from build123d import *

# Parameters (mm, degrees)
BASE_PLATE_PROFILE_SKETCH_R   = 6
BASE_PLATE_PROFILE_SKETCH_R_2 = 5
BASE_PLATE_PROFILE_SKETCH_R_3 = 9.5
BASE_PLATE_14MM_DEPTH         = 14
INTERLOCKING_RAILS_SKETCH_W   = 89
INTERLOCKING_RAILS_SKETCH_H   = 9
INTERLOCKING_RAILS_SKETCH_W_2 = 27
INTERLOCKING_RAILS_SKETCH_H_2 = 19
INTERLOCKING_RAILS_SKETCH_W_3 = 18
INTERLOCKING_RAILS_32MM_DEPTH = 32
RAIL_SLOT_CUT_REACH           = 205.941


with BuildPart() as part:
    # Base Plate Profile Sketch → Base Plate 14mm (new body)
    with BuildSketch(Plane(origin=(0, 0, 0), x_dir=(1, 0, 0), z_dir=(0, 1, 0))):
        with BuildLine():
            Line((0, 0), (-117.109003688, 0))
            ThreePointArc((-117.109003688, 0), (-123.536879785, 2.339555569), (-126.957081218, 8.263518223))
            Line((-126.957081218, 8.263518223), (-139.9366539, 81.874332802))
            ThreePointArc((-139.9366539, 81.874332802), (-135.998914322, 96.570176974), (-122.210114346, 103))
            Line((-122.210114346, 103), (-56.522720755, 103))
            ThreePointArc((-56.522720755, 103), (-49.311103576, 105.408723877), (-44.994618812, 111.667903721))
            Line((-44.994618812, 111.667903721), (-38.331477751, 134.720469728))
            ThreePointArc((-38.331477751, 134.720469728), (-19.616213283, 146.832039713), (-5, 130))
            Line((-5, 130), (-5, 77.5))
            Line((-5, 77.5), (0, 55))
            Line((0, 55), (0, 0))
        make_face()
        with Locations(Location((-22, 130, 0), (0, 0, 270))):
            Circle(BASE_PLATE_PROFILE_SKETCH_R, mode=Mode.SUBTRACT)
        with Locations(Location((-122.210114346, 85, 0), (0, 0, 270))):
            Circle(BASE_PLATE_PROFILE_SKETCH_R_2, mode=Mode.SUBTRACT)
        with Locations(Location((-90.210114346, 79.5, 0), (0, 0, 270))):
            Circle(BASE_PLATE_PROFILE_SKETCH_R_3, mode=Mode.SUBTRACT)
        with Locations(Location((-28.210114346, 79.5, 0), (0, 0, 270))):
            Circle(BASE_PLATE_PROFILE_SKETCH_R_3, mode=Mode.SUBTRACT)
    extrude(amount=BASE_PLATE_14MM_DEPTH)

    # Interlocking Rails Sketch → Interlocking Rails 32mm (add)
    with BuildSketch(Plane(origin=(0, 0, 0), x_dir=(1, 0, 0), z_dir=(0, 1, 0))):
        with Locations((-49.5, 4.5)):
            Rectangle(INTERLOCKING_RAILS_SKETCH_W, INTERLOCKING_RAILS_SKETCH_H)
        with Locations((-80.5, 27.5)):
            Rectangle(INTERLOCKING_RAILS_SKETCH_W_2, INTERLOCKING_RAILS_SKETCH_H_2)
        with Locations((-49.5, 50.5)):
            Rectangle(INTERLOCKING_RAILS_SKETCH_W, INTERLOCKING_RAILS_SKETCH_H)
        with Locations((-4.5, 27.5)):
            Rectangle(INTERLOCKING_RAILS_SKETCH_W_3, INTERLOCKING_RAILS_SKETCH_H_2)
    extrude(amount=INTERLOCKING_RAILS_32MM_DEPTH)

    # Rail Slot Sketch → Rail Slot Cut (cut, up to next)
    with BuildSketch(Plane(origin=(0, 14, 0), x_dir=(1, 0, 0), z_dir=(0, 1, 0)), mode=Mode.PRIVATE) as rail_slot_cut_sk1:
        Polygon((-81.5, 46), (-81.5, 37), (-67, 37), (-67, 18), (-81.5, 18), (-81.5, 9), (-21.5, 9), (-21.5, 46), align=None)
    rail_slot_cut_tool1 = extrude(rail_slot_cut_sk1.sketch, amount=-RAIL_SLOT_CUT_REACH, mode=Mode.PRIVATE) & part.part
    add(rail_slot_cut_tool1.solids().sort_by_distance((-48.276742, 14, -27.5))[0], mode=Mode.SUBTRACT)


solid = part.part
Could you check a few things on this model? Use its own coordinates, in mm. A direction names the side the tool comes from. Coordinates: 2 decimals unless noted, no trailing zeros. Order: outer loops, then holes, each group sorted by start corner. A loop starts at its lowest first (then second) coordinate and runs counter-clockwise, first axis right, second up.
Q1. Suppose I cut it at A-A on y = 24. Please give me the cut outline in (x, z).
Q2. Please list where these lines run through material, in increasing order: L1, parallel to Z at x = -72.5, y = 7.5; L2, parallel to Z at x = -71, y = 16.5; L3, parallel to Z at x = -50, y = 21.
Q3. Which directions (+Z, -Z, +X, -X, +Y, -Y) give clear straight access to the entire face, cutting with the end or side of a thin tool? Please do faces 1 (the flat face through (-94, 23, -4)), 2 (the flat face through (-5, 23, -4)), 3 (the flat face through (-50, 16, -46)).
Q4. Suppose I cut it at B-B on z = -42.5. Please give me the cut outline in (x, y), and give its area (3 significant figures).
Q5. Suppose I cut it at C-C on x = -52. Please give me the cut outline in (y, z).
Q6. Thinking about a two-plate mould opening in X: for faces 4 (the cylindrical face through (-19.954, 6.902, -146.876)), 5 (the flat face through (-50, 16, -9)), 6 (the flat face through (4.5, 16, -27)), which applies, released by +X, released by -X, zero draft, split by the parting line, or undercut?
Q7. Suppose I cut it at D-D on z = -85. Please give me the cut outline in (x, y), and give its area (3 significant figures).
Q8. Will these pins go through, and if not, where does the flat tip stop? pin 1 (1.5 mm diameter, centred on x = -14, z = -106, fed in from +Y); pin 2 (4.5 mm diameter, centred on y = 23, z = -48.5, fed in from +X); pin 3 (10 mm diameter, centred on x = -24.5, y = 13, fed in from +Z); pin 4 (15.5 mm diameter, centred on y = 6, z = -6, fed in from +X).
Answer:
1. outline: (-94, -55) - (-5, -55) - (-5, -46) - (-94, -46) - close; (-94, -37) - (-67, -37) - (-67, -18) - (-94, -18) - close; (-94, -9) - (-5, -9) - (-5, 0) - (-94, 0) - close; (-13.5, -37) - (4.5, -37) - (4.5, -18) - (-13.5, -18) - close
2. L1: z = -103 to -46, -37 to -18, -9 to 0
2. L2: z = -55 to -46, -37 to -18, -9 to 0
2. L3: z = -55 to -46, -9 to 0
3. face 1: +Z, -Z, -X, +Y
3. face 2: +Z, +X, +Y
3. face 3: +Y
4. outline: (-132.99, 0) - (-81.5, 0) - (-81.5, 14) - (-132.99, 14) - close; (-21.5, 0) - (0, 0) - (0, 14) - (-21.5, 14) - close
4. area: 1,020 mm2
5. outline: (0, -103.88) - (14, -103.88) - (14, -55) - (32, -55) - (32, -46) - (0, -46) - close; (0, -9) - (32, -9) - (32, 0) - (0, 0) - close
6. face 4: split by the parting line
6. face 5: undercut
6. face 6: released by +X
7. outline: (-140.21, 0) - (-127.21, 0) - (-127.21, 14) - (-140.21, 14) - close; (-117.21, 0) - (-97.96, 0) - (-97.96, 14) - (-117.21, 14) - close; (-82.46, 0) - (-35.96, 0) - (-35.96, 14) - (-82.46, 14) - close; (-20.46, 0) - (-5, 0) - (-5, 14) - (-20.46, 14) - close
7. area: 1,320 mm2
8. pin 1: stops at y = 14
8. pin 2: stops at x = -5
8. pin 3: stops at z = 0
8. pin 4: stops at x = 0
